from build123d import *

# Parameters (mm, degrees)
BUSHING_BODY_DEPTH          = 14
FRONT_PIVOT_PIN_PROFILE_6_R = 3
FRONT_PIVOT_PIN_6_DEPTH     = 2.5
REAR_START                  = 2.5
REAR_PIVOT_PIN_PROFILE_6_R  = 3
REAR_PIVOT_PIN_6_DEPTH      = 2.5
CROSS_COUNTERBORE_PROFILE_R = 5
CROSS_COUNTERBORE_DEPTH     = 4
CROSS_HOLE_PROFILE_6_R      = 3
CROSS_HOLE_6_DEPTH          = 16


with BuildPart() as part:
    # Body Profile Ø19 D-Flat → Bushing Body (new body)
    with BuildSketch(Plane.XY):
        with BuildLine():
            Line((8, 5.123475383), (8, -5.123475383))
            ThreePointArc((8, -5.123475383), (-9.5, 0), (8, 5.123475383))
        make_face()
    extrude(amount=BUSHING_BODY_DEPTH)

    # Front Pivot Pin Profile Ø6 → Front Pivot Pin Ø6 (add)
    with BuildSketch(Plane.XY.offset(14)):
        Circle(FRONT_PIVOT_PIN_PROFILE_6_R)
    extrude(amount=FRONT_PIVOT_PIN_6_DEPTH)

    # Rear Pivot Pin Profile Ø6 → Rear Pivot Pin Ø6 (add)
    with BuildSketch(Plane(origin=(0, 0, 0), x_dir=(-1, 0, 0), z_dir=(0, 0, -1)).offset(REAR_START)):
        with Locations(Location((0, 0, 0), (0, 0, 180))):
            Circle(REAR_PIVOT_PIN_PROFILE_6_R)
    extrude(amount=-REAR_PIVOT_PIN_6_DEPTH)

    # Cross Counterbore Profile → Cross Counterbore (cut)
    with BuildSketch(Plane(origin=(0, 10, 0), x_dir=(1, 0, 0), z_dir=(0, 1, 0))):
        with Locations(Location((0, -7, 0), (0, 0, 270))):
            Circle(CROSS_COUNTERBORE_PROFILE_R)
    extrude(amount=-CROSS_COUNTERBORE_DEPTH, mode=Mode.SUBTRACT)

    # Cross Hole Profile Ø6 → Cross Hole Ø6 (cut)
    with BuildSketch(Plane(origin=(0, 6, 0), x_dir=(1, 0, 0), z_dir=(0, 1, 0))):
        with Locations(Location((0, -7, 0), (0, 0, 270))):
            Circle(CROSS_HOLE_PROFILE_6_R)
    extrude(amount=-CROSS_HOLE_6_DEPTH, mode=Mode.SUBTRACT)


solid = part.part
Can you work these out from the model? Positions are in its coordinate system, mm. A direction names the side the tool comes from. Give positions to 0.01 mm unless a question says otherwise; leave off trailing zeros. Loops run counter-clockwise (first coordinate to the right, second up) from the corner with the lowest first, then second, coordinate; pieces in that order, holes last. Notation, with made-up numbers: (19.25, -32.75) - (63.25, -32.75) arc R23 ccw to (63.25, -7.75) - close; hole circle Ø5 at (-19, 62). An arc over 180 degrees is marked (long way). Answer as a JSON object with one key per item and string values.
Q1. Imagine slicing it at A-A on x = 0. Write out the boundary of the cut face in (y, z), plus the area to 3 significant figures.
Geometry says:
{"outline": "(-9.5, 0) - (-3, 0) - (-3, -2.5) - (3, -2.5) - (3, 0) - (9.5, 0) - (9.5, 2) - (6, 2) - (6, 4) - (-9.5, 4) - close; (-9.5, 10) - (6, 10) - (6, 12) - (9.5, 12) - (9.5, 14) - (3, 14) - (3, 16.5) - (-3, 16.5) - (-3, 14) - (-9.5, 14) - close", "area": "168 mm²"}
Q2. Imagine slicing it at C-C on z = 7. Write out the boundary of the cut face in (x, y), plus the area to 3 significant figures.
Geometry says:
{"outline": "(-5, 6) - (-5, 8.08) arc R9.5 ccw to (-3, -9.01) - (-3, 6) - close; (3, -9.01) arc R9.5 ccw to (8, -5.12) - (8, 5.12) arc R9.5 ccw to (5, 8.08) - (5, 6) - (3, 6) - close", "area": "151 mm²"}
Q3. Imagine slicing it at D-D on x = 3.5. Write out the boundary of the cut face in (y, z), plus the area to 3 significant figures.
Geometry says:
{"outline": "(-8.83, 0) - (8.83, 0) - (8.83, 3.43) - (6, 3.43) - (6, 10.57) - (8.83, 10.57) - (8.83, 14) - (-8.83, 14) - close", "area": "227 mm²"}
Q4. If I drill on L1, parallel to Z at x = 0, y = 5; L2, parallel to Z at x = 0, y = 0.5; L3, parallel to Z at x = -5, y = -1, over which ranges is the centre line in solid material (lowest first)?
Geometry says:
{"L1": "0 to 4, 10 to 14", "L2": "-2.5 to 4, 10 to 16.5", "L3": "0 to 14"}
Q5. Imagine slicing it at B-B on y = 0. Write out the boundary of the cut face in (x, z).
Geometry says:
{"outline": "(-9.5, 0) - (-3, 0) - (-3, -2.5) - (3, -2.5) - (3, 0) - (8, 0) - (8, 14) - (3, 14) - (3, 16.5) - (-3, 16.5) - (-3, 14) - (-9.5, 14) - close; hole circle Ø6 at (0, 7)"}
Q6. Which directions (+Z, -Z, +X, -X, +Y, -Y) give clear straight access to the entire face, cutting with the end or side of a thin tool? Please do faces 4 (the flat face through (-3, -2, 14)), 5 (the cylindrical face through (-1.15, -1.64, 9.77)), 6 (the flat face through (0, 0, -2.5)), 7 (the flat face through (-3, -2, 0)), 8 (the flat face through (0.1, 6, 10.3)).
Geometry says:
{"face 4": "+Z", "face 5": "+Y, -Y", "face 6": "-Z, +X, -X, +Y, -Y", "face 7": "-Z", "face 8": "+Y"}
Q7. Will these pins go through, and if not, where does the flat tip stop? P1, Ø5, axis at y = 4, z = 14, coming from the -X side; P2, Ø1, axis at x = -3.5, y = 7.5, coming from the -Z side; P3, Ø5, axis at x = 0, z = 7, coming from the +Y side; P4, Ø1.5, axis at x = 4, z = 7.5, coming from the +Y side.
Geometry says:
{"P1": "x = -9.38", "P2": "z = 0", "P3": "through", "P4": "y = 6"}
Q8. If we mould it in two halves opening along X, with no side actions, what happens to faces 1 (the flat face through (0, 0, 16.5)), 2 (the cylindrical face through (-3, 7, 3)), 3 (the cylindrical face through (2.86, -0.9, -1.27))? For each: pulls with the +X half, pulls with the -X half, needs draft (parallel to the pull), parting line crosses it, or undercut.
Geometry says:
{"face 1": "needs draft", "face 2": "undercut", "face 3": "parting line crosses it"}
